```python
from build123d import *

# Parameters (mm, degrees)
SKETCH_1_W          = 40
SKETCH_1_H          = 410
EXTRUDE_1_DEPTH     = 20
SKETCH_2_W          = 16
SKETCH_2_H          = 410
CUT_EXTRUDE_1_DEPTH = 10
SKETCH_3_W          = 20
SKETCH_3_H          = 38
SKETCH_3_H_2        = 30
CUT_EXTRUDE_2_DEPTH = 7
SKETCH_4_W          = 20
SKETCH_4_H          = 30
SKETCH_4_H_2        = 38
CUT_EXTRUDE_3_DEPTH = 7
HOLE_WIZARD_M4_1_D  = 3.3
CHAMFER_1_SIZE      = 0.5


with BuildPart() as part:
    # 草图1 → 凸台-拉伸1 (new body)
    with BuildSketch(Plane(origin=(0, 0, 0), x_dir=(0, 0, -1), z_dir=(1, 0, 0))):
        Rectangle(SKETCH_1_W, SKETCH_1_H)
    extrude(amount=EXTRUDE_1_DEPTH)

    # 草图2 → 切除-拉伸1 (cut)
    with BuildSketch(Plane.ZY):
        Rectangle(SKETCH_2_W, SKETCH_2_H)
    extrude(amount=-CUT_EXTRUDE_1_DEPTH, mode=Mode.SUBTRACT)

    # 草图3 → 切除-拉伸2 (cut)
    with BuildSketch(Plane.XY.offset(20)):
        with Locations((10, -186)):
            Rectangle(SKETCH_3_W, SKETCH_3_H)
        with Locations((10, 48)):
            Rectangle(SKETCH_3_W, SKETCH_3_H_2)
    extrude(amount=-CUT_EXTRUDE_2_DEPTH, mode=Mode.SUBTRACT)

    # 草图4 → 切除-拉伸3 (cut)
    with BuildSketch(Plane(origin=(0, 0, -20), x_dir=(-1, 0, 0), z_dir=(0, 0, -1))):
        with Locations((-10, 48)):
            Rectangle(SKETCH_4_W, SKETCH_4_H)
        with Locations((-10, -186)):
            Rectangle(SKETCH_4_W, SKETCH_4_H_2)
    extrude(amount=-CUT_EXTRUDE_3_DEPTH, mode=Mode.SUBTRACT)

    # M4 螺纹孔1 (through all)
    with Locations(Plane(origin=(0, 0, -13), x_dir=(-1, 0, 0), z_dir=(0, 0, -1))):
        with Locations((-15, 55.5), (-15, 40.5), (-15, -174.49792687), (-15, -189.49792687)):
            Hole(HOLE_WIZARD_M4_1_D / 2)

    # 倒角1
    chamfer_1_edges = [part.edges().sort_by_distance(p)[0] for p in [
        (20, 134, 20),
        (0, -205, -10.5),
        (0, 205, 14),
        (5, 205, 8),
        (10, -205, 0),
        (5, -205, 8),
        (5, -205, -8),
        (10, 205, 0),
        (5, 205, -8),
        (0, 0, 8),
        (0, 0, -8),
        (20, -205, 0),
        (0, -205, 10.5),
        (0, -186, 13),
        (0, -167, 16.5),
        (20, -186, 13),
        (20, -167, 16.5),
        (10, -205, 13),
        (10, -167, 20),
        (20, -67, 20),
        (0, -67, 20),
        (0, 48, 13),
        (0, 33, 16.5),
        (0, 63, 16.5),
        (20, 48, 13),
        (20, 63, 16.5),
        (20, 33, 16.5),
        (0, 134, 20),
        (10, 33, 20),
        (10, 63, 20),
        (0, 205, -14),
        (0, 134, -20),
        (20, 134, -20),
        (0, 48, -13),
        (0, 63, -16.5),
        (0, 33, -16.5),
        (20, 48, -13),
        (20, 33, -16.5),
        (20, 63, -16.5),
        (10, 63, -20),
        (10, 33, -20),
        (20, 205, 0),
        (0, -67, -20),
        (20, -67, -20),
        (10, 205, 20),
        (0, -186, -13),
        (0, -167, -16.5),
        (10, 205, -20),
        (10, -205, -13),
        (20, -186, -13),
        (20, -167, -16.5),
        (10, -167, -20),
    ]]
    chamfer(chamfer_1_edges, length=CHAMFER_1_SIZE)


solid = part.part
```
Input: part model. Units: mm. Frame: model coordinates. A direction names the side the tool comes from. Coordinates: 2 decimals unless noted, no trailing zeros. Order: outer loops, then holes, each group sorted by start corner. A loop starts at its lowest first (then second) coordinate and runs counter-clockwise, first axis right, second up. Notation, with made-up numbers: (-4.75, 10) - (17.25, 10) arc R36 ccw to (17.25, 48) - close; hole circle Ø9 at (21, -11.75). An arc over 180 degrees is marked (long way). Put each result on its own line as item: value.
1. Contact query for flat-ended pins moving along their axis: pin 1 Ø2 at (x, z) = (5.5, 15) entering from -Y; pin 2 Ø9.5 at (x, y) = (14, 42) entering from +Z; pin 3 Ø5 at (y, z) = (85, 2) entering from -X. Output: stop coordinate, or through.
Report:
pin 1: stops at y = -167
pin 2: stops at z = 13
pin 3: stops at x = 10
2. Reachability of faces 1 (the face through (10, -185, -13)), 2 (the face through (10, 63, 16)), 3 (the face through (10, -185, 13)), 4 (the face through (10, 48, -13)) from +Z, -Z, +X, -X, +Y, -Y: full face, straight path, thin tool, end or side. Return the list, or none.
Report:
face 1: -Z, +X, -X, -Y
face 2: +Z, +X, -X
face 3: +Z, +X, -X, -Y
face 4: -Z, +X, -X
3. Cut plane A-A on y = -117.5. Return the cut outline in (x, z).
Report:
outline: (0, -19.5) - (0.5, -20) - (19.5, -20) - (20, -19.5) - (20, 19.5) - (19.5, 20) - (0.5, 20) - (0, 19.5) - (0, 8.5) - (0.5, 8) - (10, 8) - (10, -8) - (0.5, -8) - (0, -8.5) - close
4. Draft query along Y for faces 5 (the face through (5, -3, -8)), 6 (the face through (10, -167, 16)), 7 (the face through (10, 63, -16)). Return one class per face: pulls with the +Y half, pulls with the -Y half, needs draft (parallel to the pull), parting line crosses it, or undercut.
Report:
face 5: needs draft
face 6: pulls with the -Y half
face 7: undercut
5. Line query: line 1 along Y through (x, z) = (15, -4.5); line 2 along Y through (x, z) = (14.5, 5); line 3 along Z through (x, y) = (8.75, 151.5). Output: solid intervals per line, ascending.
Report:
line 1: y = -205 to -191.15, -187.85 to -176.15, -172.85 to 38.85, 42.15 to 53.85, 57.15 to 205
line 2: y = -205 to -191.07, -187.93 to -176.07, -172.93 to 38.93, 42.07 to 53.93, 57.07 to 205
line 3: z = -20 to -8, 8 to 20
